Input: part model. Units: mm. Frame: model coordinates. A direction names the side the tool comes from. Coordinates: 2 decimals unless noted, no trailing zeros. Write each loop counter-clockwise with the first axis right and the second up, starting at its lowest first coordinate (ties: lowest second). Pieces come first, ordered by that corner, then holes.
1) Section query A-A (y = -13.25). Output: boundary loops of the cut face in (x, z), then the cut area to 3 significant figures.
2) Set-up query: faces 1 (the cylindrical face through (-38.14, -16.9, -0.21)), 2 (the cylindrical face through (20.71, -17.1, -0.22)). Return all of +Z, -Z, +X, -X, +Y, -Y with unobstructed straight access to the full face (end or side cutting, diameter ignored); none if empty.
3) Pin query (flat end, axial travel): pin 1 Ø6 at (x, y) = (42, -15.5) entering from -Z; pin 2 Ø3 at (x, z) = (23.5, 4) entering from +Y; pin 3 Ø3 at (x, z) = (38, 3.5) entering from +Y. Return the tip coordinate at first contact, or that it passes through.
4) Line query: L1, parallel to Y at x = -9.5, z = -1.5; L2, parallel to Y at x = -30, z = 3.25; L3, parallel to Z at x = 26, y = -13.75. Output: solid intervals per line, ascending.
5) Section query C-C (x = -14.5). Output: boundary loops of the cut face in (y, z), then the cut area to 3 significant figures.
6) Section query B-B (z = -2.25). Output: boundary loops of the cut face in (x, y), then the cut area to 3 significant figures.
from build123d import *


with BuildPart() as part:
    # Sketch1 → Revolve1 (revolve)
    with BuildSketch(Plane.XY):
        Polygon((-57.596279733, -12.106542056), (-57.596279733, -7.106542056), (-38.696279733, -7.106542056), (-38.696279733, -7.306542056), (-37.596279733, -7.306542056), (-37.596279733, -7.106542056), (77.403720267, -7.106542056), (77.403720267, -7.306542056), (78.503720267, -7.306542056), (78.503720267, -7.106542056), (97.403720267, -7.106542056), (97.403720267, -12.106542056), align=None)
    revolve(axis=Axis((97.403720267, -12.106542056, 0), (-1, 0, 0)))


solid = part.part
Answer:
1. outline: (-57.6, -4.87) - (-38.7, -4.87) - (-38.7, -4.66) - (-37.6, -4.66) - (-37.6, -4.87) - (77.4, -4.87) - (77.4, -4.66) - (78.5, -4.66) - (78.5, -4.87) - (97.4, -4.87) - (97.4, 4.87) - (78.5, 4.87) - (78.5, 4.66) - (77.4, 4.66) - (77.4, 4.87) - (-37.6, 4.87) - (-37.6, 4.66) - (-38.7, 4.66) - (-38.7, 4.87) - (-57.6, 4.87) - close
1. area: 1,510 mm2
2. face 1: none
2. face 2: +X, -X
3. pin 1: stops at z = -4.98
3. pin 2: stops at y = -7.78
3. pin 3: stops at y = -7.52
4. L1: y = -16.88 to -7.34
4. L2: y = -15.91 to -8.31
4. L3: z = -4.72 to 4.72
5. outline: circle Ø10 at (-12.11, 0)
5. area: 78.5 mm2
6. outline: (-57.6, -16.57) - (-38.7, -16.57) - (-38.7, -16.35) - (-37.6, -16.35) - (-37.6, -16.57) - (77.4, -16.57) - (77.4, -16.35) - (78.5, -16.35) - (78.5, -16.57) - (97.4, -16.57) - (97.4, -7.64) - (78.5, -7.64) - (78.5, -7.87) - (77.4, -7.87) - (77.4, -7.64) - (-37.6, -7.64) - (-37.6, -7.87) - (-38.7, -7.87) - (-38.7, -7.64) - (-57.6, -7.64) - close
6. area: 1,380 mm2
